```python
from build123d import *

# Parameters (mm, degrees)
DRIVE_WHEEL_PROFILE_R           = 47.5
DRIVE_WHEEL_PROFILE_R_2         = 5
DRIVE_DISC_95_DEPTH             = 5
LOCKING_START                   = 5
SKETCH1_3_R                     = 5
SKETCH1_3_R_2                   = 5.3
LOCKING_HUB_AND_DRIVE_PIN_DEPTH = 5


with BuildPart() as part:
    # Drive Wheel Profile → Drive Disc _95 (new body)
    with BuildSketch(Plane.XY):
        Circle(DRIVE_WHEEL_PROFILE_R)
        Circle(DRIVE_WHEEL_PROFILE_R_2, mode=Mode.SUBTRACT)
    extrude(amount=-DRIVE_DISC_95_DEPTH)

    # Sketch1_3 → Locking Hub and Drive Pin (add)
    # profile 1 of 2: a face of its own
    with BuildSketch(Plane.XY.offset(LOCKING_START)):
        with BuildLine():
            ThreePointArc((-19.989232296, -18.150222925), (-12.978464592, 0), (-19.989232296, 18.150222925))
            ThreePointArc((-19.989232296, 18.150222925), (27, 0), (-19.989232296, -18.150222925))
        make_face()
        Circle(SKETCH1_3_R, mode=Mode.SUBTRACT)
    # profile 2 of 2: a face of its own
    with BuildSketch(Plane.XY.offset(LOCKING_START)):
        with Locations((-39, 0)):
            Circle(SKETCH1_3_R_2)
    extrude(amount=-LOCKING_HUB_AND_DRIVE_PIN_DEPTH)


solid = part.part
```
Work out the finished part from the listing and answer in its coordinate system (mm). A direction names the side the tool comes from. Coordinates: 2 decimals unless noted, no trailing zeros. Write each loop counter-clockwise with the first axis right and the second up, starting at its lowest first coordinate (ties: lowest second). Pieces come first, ordered by that corner, then holes.
Q1. A cutting plane is placed at A-A, the plane y = 0. Give the vertices of the cut face in (x, z).
Q2. A cutting plane is placed at C-C, the plane z = 2. Give the vertices of the cut face in (x, y), then the cut area to 3 significant figures.
Q3. Determine the mould class of faces 1 (the face through (-1.08, -4.88, 0.07)), 2 (the face through (-10.3, -46.37, -2.46)), 3 (the face through (9, 0, 5)) for opening direction X: released by +X, released by -X, zero draft, split by the parting line, or undercut.
Q4. A cutting plane is placed at B-B, the plane x = 0. Give the vertices of the cut face in (y, z), then the cut area to 3 significant figures.
Q5. Which of the six approach directions +Z, -Z, +X, -X, +Y, -Y give full straight-line access (tool end or side, diameter ignored) to faces 4 (the face through (-39, 0, 5)), 5 (the face through (-12.98, -0.28, 2.54))?
Q6. Find the intervals of material crossed by line 1 (Y direction, x = 0, z = -2.5); line 2 (Z direction, x = -34, y = 12.5); line 3 (X direction, y = 4, z = -3.5), in increasing order.
Q7. A cutting plane is placed at D-D, the plane x = -39. Give the vertices of the cut face in (y, z).
Q8. Each of these flat-tipped pins is pushed along its axis until it touches: pin 1 Ø4 at (y, z) = (-27.5, 0.5) entering from +X; pin 2 Ø5 at (x, z) = (36, -1.5) entering from +Y; pin 3 Ø8 at (x, y) = (26.5, -33) entering from +Z; pin 4 Ø1 at (x, y) = (2.5, -0.5) entering from -Z. Where does it stop, or does it pass through?
Findings below:
1. outline: (-47.5, -5) - (-5, -5) - (-5, 5) - (-12.98, 5) - (-12.98, 0) - (-33.7, 0) - (-33.7, 5) - (-44.3, 5) - (-44.3, 0) - (-47.5, 0) - close; (5, -5) - (47.5, -5) - (47.5, 0) - (27, 0) - (27, 5) - (5, 5) - close
2. outline: circle Ø10.6 at (-39, 0); (-19.99, -18.15) arc R27 ccw (long way) to (-19.99, 18.15) arc R27 cw to start; hole circle Ø10 at (0, 0)
2. area: 1,950 mm2
3. face 1: undercut
3. face 2: split by the parting line
3. face 3: zero draft
4. outline: (-47.5, -5) - (-5, -5) - (-5, 5) - (-27, 5) - (-27, 0) - (-47.5, 0) - close; (5, -5) - (47.5, -5) - (47.5, 0) - (27, 0) - (27, 5) - (5, 5) - close
4. area: 645 mm2
5. face 4: +Z, +X, -X, +Y, -Y
5. face 5: +Z
6. line 1: y = -47.5 to -5, 5 to 47.5
6. line 2: z = -5 to 0
6. line 3: x = -47.33 to -3, 3 to 47.33
7. outline: (-27.12, -5) - (27.12, -5) - (27.12, 0) - (5.3, 0) - (5.3, 5) - (-5.3, 5) - (-5.3, 0) - (-27.12, 0) - close
8. pin 1: stops at x = 40.03
8. pin 2: stops at y = 33.67
8. pin 3: stops at z = 0
8. pin 4: passes through
